Could you check a few things on this drawing? It's one solid part, dimensions in mm from its lowest x, y, z. A direction names the side the tool comes from. Round coordinates to 2 decimals unless told otherwise and drop trailing zeros. Write each loop counter-clockwise with the first axis right and the second up, starting at its lowest first coordinate (ties: lowest second). Pieces come first, ordered by that corner, then holes. Notation, with made-up numbers: (-20.75, 51) - (-12.75, 51) arc R26 ccw to (-12.75, 78) - close; hole circle Ø2 at (2, 66). An arc over 180 degrees is marked (long way). Put each result on its own line as item: value.
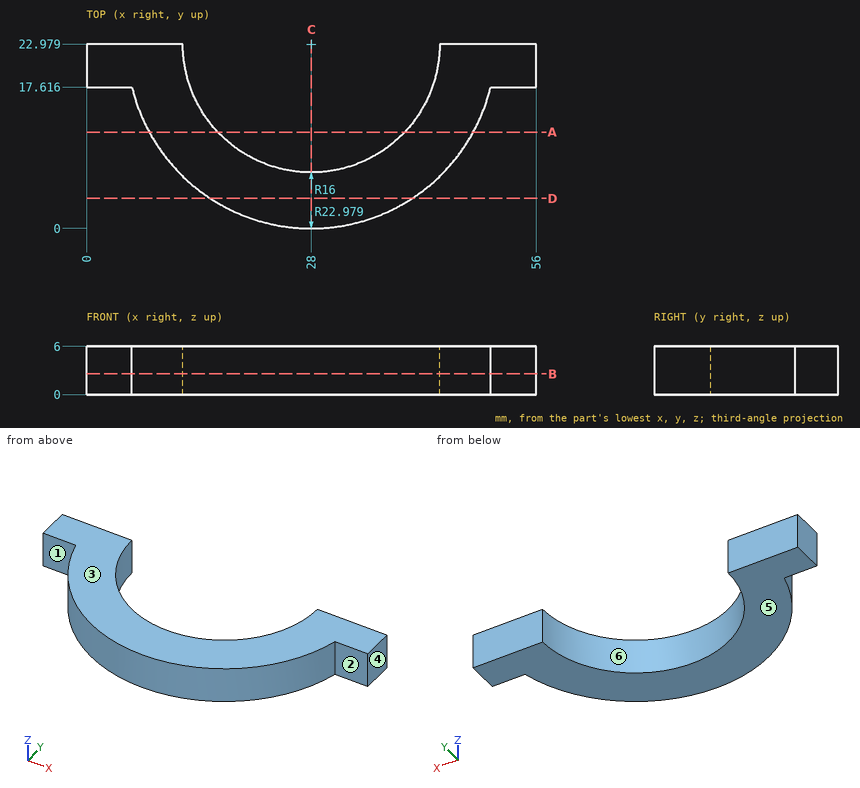
(1) For the marked faces 1, 2 and 3, which set-ups out of +Z, -Z, +X, -X, +Y, -Y let a thin tool reach every point of the face, with its end or its side?
Values found:
face 1: +Z, -Z, -X, -Y
face 2: +Z, -Z, +X, -Y
face 3: +Z, +X, -X, +Y, -Y
(2) Imagine slicing it at C-C, the plane x = 28. List the corners of the cut face in (y, z) for me, then the cut area to 3 significant figures.
Values found:
outline: (0, 0) - (6.98, 0) - (6.98, 6) - (0, 6) - close
area: 41.9 mm^2
(3) I'm going to push flat-ended pins straight in: pin 1 (1 mm diameter, centred on x = 39.5, z = 0.5, fed in from +Y); pin 2 (1.5 mm diameter, centred on x = 15, z = 4, fed in from +Y). Where does each tip first touch, or does it pass through?
Values found:
pin 1: stops at y = 12.4
pin 2: stops at y = 14.8
(4) Imagine slicing it at A-A, the plane y = 12. List the corners of the cut face in (x, z) for me.
Values found:
outline: (7.81, 0) - (16.36, 0) - (16.36, 6) - (7.81, 6) - close; (39.64, 0) - (48.19, 0) - (48.19, 6) - (39.64, 6) - close
(5) Imagine slicing it at D-D, the plane y = 3.75. List the corners of the cut face in (x, z) for me.
Values found:
outline: (15.42, 0) - (40.58, 0) - (40.58, 6) - (15.42, 6) - close
(6) Please list where these lines run through material, in increasing order: probe 1 along Y at (x, z) = (51, 4.9); probe 2 along X at (y, z) = (10.5, 3.85) (1 decimal); probe 3 along X at (y, z) = (21.75, 4). Write a range as from..to.
Values found:
probe 1: y = 17.62..22.98
probe 2: x = 8.7..18, 38..47.3
probe 3: x = 0..12.05, 43.95..56
(7) If we mould it in two halves opening along X, with no side actions, what happens to the marked faces 4, 5 and 6? For each: pulls with the +X half, pulls with the -X half, needs draft (parallel to the pull), parting line crosses it, or undercut.
Values found:
face 4: pulls with the +X half
face 5: needs draft
face 6: undercut
(8) Imagine slicing it at B-B, the plane z = 2.6. List the corners of the cut face in (x, y) for me.
Values found:
outline: (0, 17.62) - (5.66, 17.62) arc R22.98 ccw to (50.34, 17.62) - (56, 17.62) - (56, 22.98) - (44, 22.98) arc R16 cw to (12, 22.98) - (0, 22.98) - close
